Part model, mm, in its own coordinate system. Coordinates: 2 decimals unless noted, no trailing zeros. Order: outer loops, then holes, each group sorted by start corner. A loop starts at its lowest first (then second) coordinate and runs counter-clockwise, first axis right, second up. Notation, with made-up numbers: (60.25, 36.25) - (97.25, 36.25) arc R26 ccw to (97.25, 71.25) - close; hole circle Ø11 at (7, 55). An arc over 180 degrees is marked (long way). Use a Markdown table: item, result. Add a question column.
1) Drop flat-ended pins along their axis: P1, Ø2, axis at y = 6, z = -60.5, coming from the -X side; P2, Ø1.5, axis at y = 7, z = -76.5, coming from the -X side; P3, Ø1.5, axis at x = -29.5, y = 4, coming from the -Z side. Give the stop position or say it passes through.
2) Wall check: L1, parallel to Z at x = -44.5, y = 3.25; L2, parallel to X at y = 2.25, z = -119.5; L3, parallel to Z at x = -46.5, y = 2. Give the ranges that are in metal, low to high. Write a range as [from, to].
3) Saw through at C-C on x = -19. List the corners of the cut face in (y, z).
4) Saw through at A-A on y = 3.25. List the corners of the cut face in (x, z).
5) Saw through at B-B on z = -94. List the corners of the cut face in (x, y).
```python
from build123d import *

# Parameters (mm, degrees)
EXTRUDE_1_DEPTH = 8


with BuildPart() as part:
    # 草图1 → 凸台-拉伸1 (new body)
    with BuildSketch(Plane(origin=(0, 0, 0), x_dir=(1, 0, 0), z_dir=(0, 1, 0))):
        with BuildLine():
            Line((-125, 0), (0, 0))
            Line((0, 0), (0, 125))
            Line((0, 125), (-10.104211917, 125))
            ThreePointArc((-10.104211917, 125), (-45.147186258, 45.147186258), (-125, 10.104211917))
            Line((-125, 10.104211917), (-125, 0))
        make_face()
    extrude(amount=EXTRUDE_1_DEPTH)


solid = part.part
```
Results are:
| question | item | result |
|---|---|---|
| 1 | P1 | x = -32.89 |
| 1 | P2 | x = -22.96 |
| 1 | P3 | z = -65.59 |
| 2 | L1 | [-45.8, 0] |
| 2 | L2 | [-10.46, 0] |
| 2 | L3 | [-43.82, 0] |
| 3 | outline | (0, -84.4) - (8, -84.4) - (8, 0) - (0, 0) - close |
| 4 | outline | (-125, -10.1) arc R120 cw to (-10.1, -125) - (0, -125) - (0, 0) - (-125, 0) - close |
| 5 | outline | (-15.53, 0) - (0, 0) - (0, 8) - (-15.53, 8) - close |
